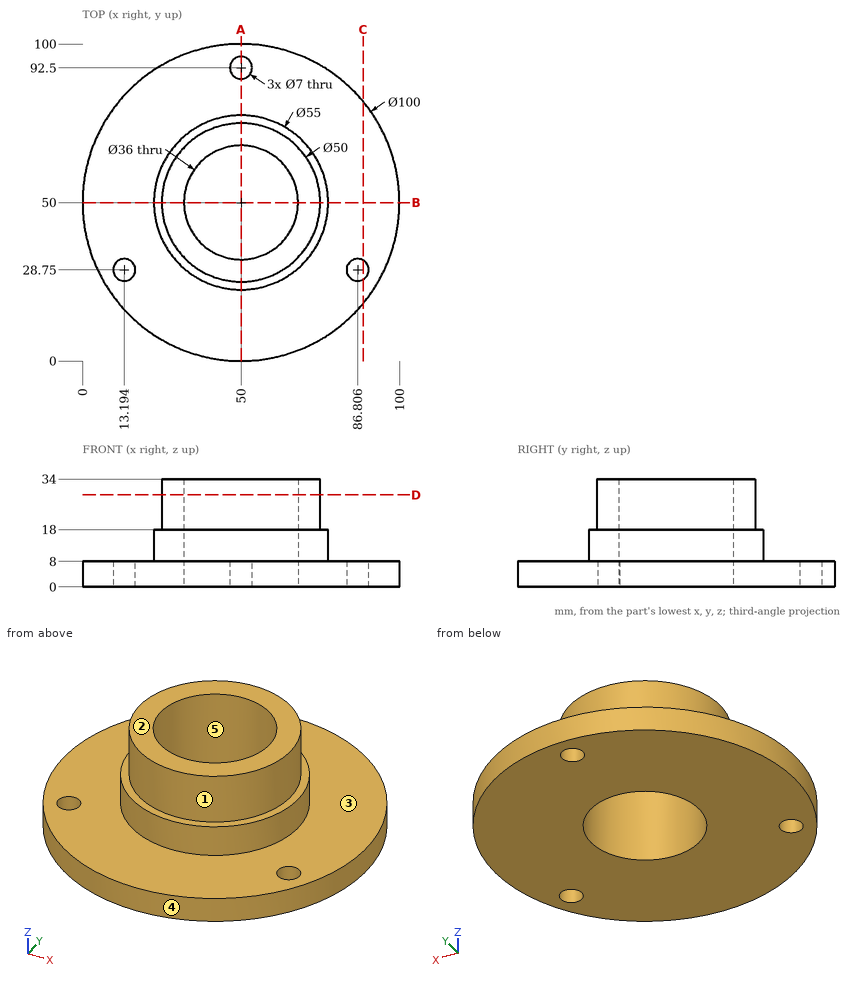
Geometry: see drawing. Coordinates: mm, zero at the bounding-box minimum. A direction names the side the tool comes from. Round coordinates to 2 decimals unless told otherwise and drop trailing zeros. Order: outer loops, then holes, each group sorted by start corner. A loop starts at its lowest first (then second) coordinate and runs counter-clockwise, first axis right, second up. Notation, with made-up numbers: (23, -4.5) - (66, -4.5) arc R18 cw to (66, 7.5) - close; hole circle Ø11 at (20.25, 39.5). An arc over 180 degrees is marked (long way). One line per question, with ' | ' between items. Start each with the question number.
1) Cut plane B-B, the plane y = 50. Return the cut outline in (x, z), then the cut area to 3 significant figures.
2) Contact query for flat-ended pins moving along their axis: P1, Ø5, axis at x = 49.5, y = 89.5, coming from the +Z side; P2, Ø3, axis at y = 28, z = 29, coming from the -X side; P3, Ø2, axis at x = 81, y = 74.5, coming from the -Z side; P4, Ø1, axis at y = 70.5, z = 24, coming from the -X side. Output: stop coordinate, or through.
3) Ray query, probe 1 along Y at (x, z) = (50, 3); probe 2 along Y at (x, z) = (50, 24); probe 3 along Z at (x, y) = (94.5, 54.5). Return the intervals inside material, ascending.
4) Set-up query: the marked faces 1 and 2. Return all of +Z, -Z, +X, -X, +Y, -Y with unobstructed straight access to the full face (end or side cutting, diameter ignored); none if empty.
5) Cut plane A-A, the plane x = 50. Return the cut outline in (y, z).
6) Pull-direction query (X, two-part tool) for the marked faces 3, 4 and 5; classes: +X half, -X half, draft (parallel to the pull), parting line (faces both ways), or undercut.
7) Cut plane C-C, the plane x = 88.5. Return the cut outline in (y, z).
8) Cut plane D-D, the plane z = 29. Return the cut outline in (x, y).
Worked out:
1) outline: (0, 0) - (32, 0) - (32, 34) - (25, 34) - (25, 18) - (22.5, 18) - (22.5, 8) - (0, 8) - close; (68, 0) - (100, 0) - (100, 8) - (77.5, 8) - (77.5, 18) - (75, 18) - (75, 34) - (68, 34) - close | area: 926 mm^2
2) P1: stops at z = 8 | P2: stops at x = 35.69 | P3: stops at z = 0 | P4: stops at x = 35
3) probe 1: y = 0 to 32, 68 to 89, 96 to 100 | probe 2: y = 25 to 32, 68 to 75 | probe 3: z = 0 to 8
4) face 1: +Z | face 2: +Z, +X, -X, +Y, -Y
5) outline: (0, 0) - (32, 0) - (32, 34) - (25, 34) - (25, 18) - (22.5, 18) - (22.5, 8) - (0, 8) - close; (68, 0) - (89, 0) - (89, 8) - (77.5, 8) - (77.5, 18) - (75, 18) - (75, 34) - (68, 34) - close; (96, 0) - (100, 0) - (100, 8) - (96, 8) - close
6) face 3: draft | face 4: parting line | face 5: undercut
7) outline: (18.1, 0) - (25.69, 0) - (25.69, 8) - (18.1, 8) - close; (31.81, 0) - (81.9, 0) - (81.9, 8) - (31.81, 8) - close
8) outline: circle Ø50 at (50, 50); hole circle Ø36 at (50, 50)
